```python
from build123d import *

# Parameters (mm, degrees)
SKETCH1_R           = 8.5
SKETCH1_R_2         = 7.1
BOSS_EXTRUDE1_DEPTH = 7
SKETCH2_W           = 5.5
SKETCH2_H           = 15
CUT_EXTRUDE1_DEPTH  = 14.910427743
CHAMFER1_SIZE       = 0.5


with BuildPart() as part:
    # Sketch1 → Boss-Extrude1 (new body)
    with BuildSketch(Plane.XY):
        Circle(SKETCH1_R)
        Circle(SKETCH1_R_2, mode=Mode.SUBTRACT)
    extrude(amount=BOSS_EXTRUDE1_DEPTH)

    # Sketch2 → Cut-Extrude1 (cut, through all)
    with BuildSketch(Plane.XY.offset(7)):
        with Locations((0, 7.5)):
            Rectangle(SKETCH2_W, SKETCH2_H)
    extrude(amount=-CUT_EXTRUDE1_DEPTH, mode=Mode.SUBTRACT)

    # Chamfer1
    chamfer1_edges = [part.edges().sort_by_distance(p)[0] for p in [
        (0, -7.1, 0),
        (0, -7.1, 7),
    ]]
    chamfer(chamfer1_edges, length=CHAMFER1_SIZE)


solid = part.part
```
Geometry check sheet. Reference: the model listing, model coordinates, mm. A direction names the side the tool comes from. Round coordinates to 2 decimals unless told otherwise and drop trailing zeros. Loops run counter-clockwise (first coordinate to the right, second up) from the corner with the lowest first, then second, coordinate; pieces in that order, holes last. Notation, with made-up numbers: (-32.75, 31) - (-27.75, 31) arc R22 cw to (-27.75, 51) - close; hole circle Ø11 at (21.25, 88.25). An arc over 180 degrees is marked (long way). Use a Markdown table: item, result.
Q1. Draft check along X on faces 3 (the flat face through (-1, -8, 0)), 4 (the cylindrical face through (-0.335, -8.493, 3.451)), 5 (the flat face through (-2.75, 7, 4)). Enter one of: released by +X, released by -X, zero draft, split by the parting line, or undercut.
Solutions:
| item | result |
|---|---|
| face 3 | zero draft |
| face 4 | split by the parting line |
| face 5 | undercut |
Q2. Cross-section at A-A on y = 0. Record the cut outline in (x, z).
Solutions:
| item | result |
|---|---|
| outline | (-8.5, 0) - (-7.6, 0) - (-7.1, 0.5) - (-7.1, 6.5) - (-7.6, 7) - (-8.5, 7) - close; (7.1, 0.5) - (7.6, 0) - (8.5, 0) - (8.5, 7) - (7.6, 7) - (7.1, 6.5) - close |
Q3. Material ranges on line 1 (X direction, y = 0, z = 2.05); line 2 (X direction, y = 7.5, z = 3.5); line 3 (Y direction, x = 0, z = 1.9), recorded low to high.
Solutions:
| item | result |
|---|---|
| line 1 | x = -8.5 to -7.1, 7.1 to 8.5 |
| line 2 | x = -4 to -2.75, 2.75 to 4 |
| line 3 | y = -8.5 to -7.1 |
Q4. Access from +Z, -Z, +X, -X, +Y, -Y to the whole of each face (thin tool, end or side, straight path). Record for faces 1 (the flat face through (2.75, 7, 4)), 2 (the conical face through (0.281, -7.237, 6.642)).
Solutions:
| item | result |
|---|---|
| face 1 | +Z, -Z, +Y |
| face 2 | +Z |
Q5. Cross-section at C-C on z = 5.75. Record the cut outline in (x, y).
Solutions:
| item | result |
|---|---|
| outline | (-2.75, 6.55) - (-2.75, 8.04) arc R8.5 ccw (long way) to (2.75, 8.04) - (2.75, 6.55) arc R7.1 cw (long way) to start |
Q6. Cross-section at B-B on x = 0. Record the cut outline in (y, z).
Solutions:
| item | result |
|---|---|
| outline | (-8.5, 0) - (-7.6, 0) - (-7.1, 0.5) - (-7.1, 6.5) - (-7.6, 7) - (-8.5, 7) - close |
Q7. Go/stop test with flat-tipped pins: P1, Ø0.7, axis at y = 7, z = 4.5, coming from the -X side; P2, Ø4, axis at y = -2.5, z = 2.5, coming from the -X side; P3, Ø3, axis at y = 2.5, z = 5, coming from the -X side; P4, Ø3, axis at x = -4, y = 3, coming from the +Z side. Record where each tip stops, or that it passes through.
Solutions:
| item | result |
|---|---|
| P1 | stops at x = -5.29 |
| P2 | stops at x = -8.49 |
| P3 | stops at x = -8.44 |
| P4 | passes through |
